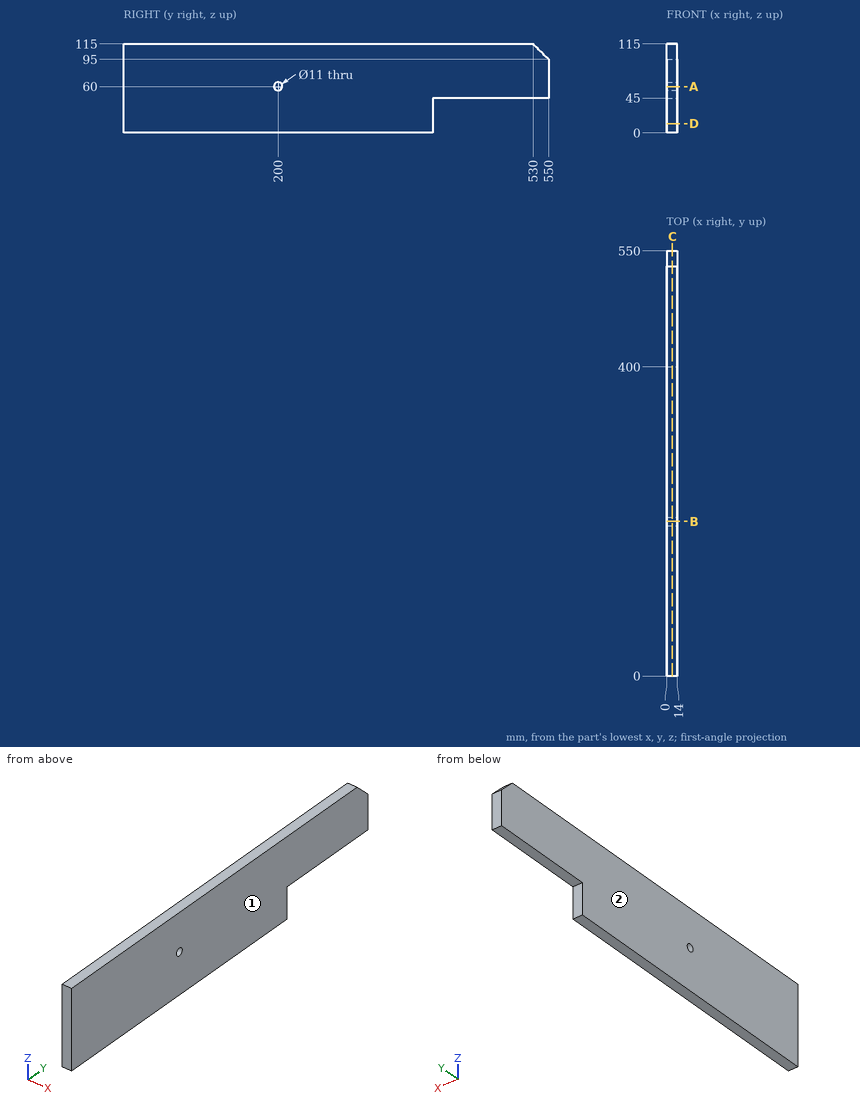
Geometry check sheet. Reference: drawing and pictorial views, mm from the part's lowest x, y, z. Give positions to 0.01 mm unless a question says otherwise; leave off trailing zeros. Write each loop counter-clockwise with the first axis right and the second up, starting at its lowest first coordinate (ties: lowest second). Pieces come first, ordered by that corner, then holes. Notation, with made-up numbers: (56.5, -27) - (108.5, -27) arc R28 cw to (108.5, -8) - close; hole circle Ø3 at (86, 14.25). An arc over 180 degrees is marked (long way). Use a Markdown table: item, result.
Q1. Thickness scan on L1, parallel to Z at x = 7.5, y = 200; L2, parallel to Y at x = 10.75, z = 60; L3, parallel to Y at x = 13, z = 35.5. Record the ranges inside material, lowest first. Write a range as [from, to].
Computed:
| item | result |
|---|---|
| L1 | z = [0, 54.5], [65.5, 115] |
| L2 | y = [0, 194.5], [205.5, 550] |
| L3 | y = [0, 400] |
Q2. Section check B-B, the plane y = 200. Enter the section's corners in (x, z).
Computed:
| item | result |
|---|---|
| outline | (0, 0) - (14, 0) - (14, 54.5) - (0, 54.5) - close; (0, 65.5) - (14, 65.5) - (14, 115) - (0, 115) - close |
Q3. Section check C-C, the plane x = 7.5. Enter the section's corners in (y, z).
Computed:
| item | result |
|---|---|
| outline | (0, 0) - (400, 0) - (400, 45) - (550, 45) - (550, 95) - (530, 115) - (0, 115) - close; hole circle Ø11 at (200, 60) |
Q4. Draft check along X on the marked faces 1 and 2. Enter one of: pulls with the +X half, pulls with the -X half, needs draft (parallel to the pull), parting line crosses it, or undercut.
Computed:
| item | result |
|---|---|
| face 1 | pulls with the +X half |
| face 2 | pulls with the -X half |
Q5. Section check A-A, the plane z = 60. Enter the section's corners in (x, y).
Computed:
| item | result |
|---|---|
| outline | (0, 0) - (14, 0) - (14, 194.5) - (0, 194.5) - close; (0, 205.5) - (14, 205.5) - (14, 550) - (0, 550) - close |
Q6. Go/stop test with a flat-tipped pin: P1, Ø7, axis at x = 9, y = 446, coming from the -Z side. Record where the tip stops, or that it passes through.
Computed:
| item | result |
|---|---|
| P1 | stops at z = 45 |
Q7. Section check D-D, the plane z = 12. Enter the section's corners in (x, y), then the cut area to 3 significant figures.
Computed:
| item | result |
|---|---|
| outline | (0, 0) - (14, 0) - (14, 400) - (0, 400) - close |
| area | 5,600 mm² |
